Here's how the part is built. I have some questions about the finished solid (model axes, mm). Coordinates: 2 decimals unless noted, no trailing zeros. Loops run counter-clockwise (first coordinate to the right, second up) from the corner with the lowest first, then second, coordinate; pieces in that order, holes last.
```python
from build123d import *

# Parameters (mm, degrees)
SKETCH1_W             = 100
SKETCH1_H             = 85
BOSS_EXTRUDE1_DEPTH   = 10
M8_TAPPED_HOLE1_D     = 6.8
M8_TAPPED_HOLE1_DEPTH = 19.75
M8_TAPPED_HOLE1_TIP   = 2.042926105


with BuildPart() as part:
    # Sketch1 → Boss-Extrude1 (new body)
    with BuildSketch(Plane.XY):
        Rectangle(SKETCH1_W, SKETCH1_H)
    extrude(amount=BOSS_EXTRUDE1_DEPTH)

    # M8 Tapped Hole1
    with Locations(Plane.XY.offset(10)):
        with Locations((-35, 25), (35, 25), (35, -25), (-35, -25)):
            Hole(M8_TAPPED_HOLE1_D / 2, depth=M8_TAPPED_HOLE1_DEPTH)
            with Locations((0, 0, -(M8_TAPPED_HOLE1_DEPTH + M8_TAPPED_HOLE1_TIP / 2))):  # 118° drill point
                Cone(0, M8_TAPPED_HOLE1_D / 2, M8_TAPPED_HOLE1_TIP, mode=Mode.SUBTRACT)


solid = part.part
```
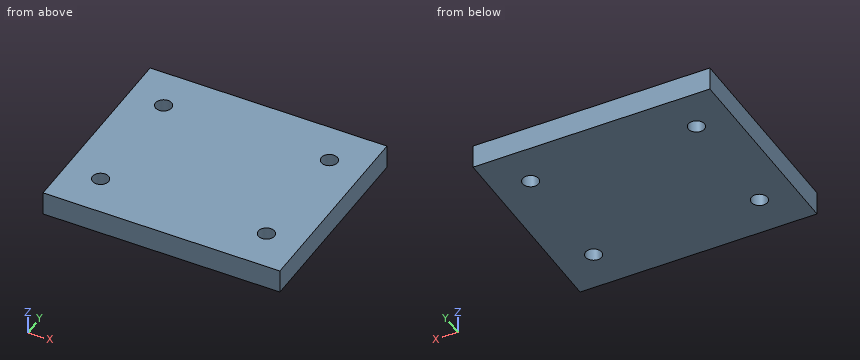
1. I want a section at C-C (z = 7.5). Please give me the cut outline in (x, y), then the cut area to 3 significant figures.
2. For pin 1 (6 mm diameter, centred on x = -35, y = 25, fed in from -Z), with a flat end and sliding along its axis, tell me the tip position at first contact or that it passes through.
3. I want a section at B-B (y = -25). Please give me the cut outline in (x, z).
4. I need wall thicknesses on line 1 along Y through (x, z) = (-35, 4.5). Which ranges of the line are inside material? Lowest first, please.
5. I want a section at A-A (x = -35). Please give me the cut outline in (y, z), then the cut area to 3 significant figures.
Response values:
1. outline: (-50, -42.5) - (50, -42.5) - (50, 42.5) - (-50, 42.5) - close; hole circle Ø6.8 at (-35, -25); hole circle Ø6.8 at (-35, 25); hole circle Ø6.8 at (35, -25); hole circle Ø6.8 at (35, 25)
1. area: 8,350 mm2
2. pin 1: passes through
3. outline: (-50, 0) - (-38.4, 0) - (-38.4, 10) - (-50, 10) - close; (-31.6, 0) - (31.6, 0) - (31.6, 10) - (-31.6, 10) - close; (38.4, 0) - (50, 0) - (50, 10) - (38.4, 10) - close
4. line 1: y = -42.5 to -28.4, -21.6 to 21.6, 28.4 to 42.5
5. outline: (-42.5, 0) - (-28.4, 0) - (-28.4, 10) - (-42.5, 10) - close; (-21.6, 0) - (21.6, 0) - (21.6, 10) - (-21.6, 10) - close; (28.4, 0) - (42.5, 0) - (42.5, 10) - (28.4, 10) - close
5. area: 714 mm2
